Verification items for the finished model (mm, model axes). Face numbers are marked on the shaded views. A direction names the side the tool comes from. Give positions to 0.01 mm unless a question says otherwise; leave off trailing zeros. Order: outer loops, then holes, each group sorted by start corner. A loop starts at its lowest first (then second) coordinate and runs counter-clockwise, first axis right, second up. Notation, with made-up numbers: (16.5, 6.5) -> (70.5, 6.5) arc R22 ccw to (70.5, 13.5) -> close; hole circle Ø3 at (80, 1). An arc over 180 degrees is marked (long way). One line per question, with ' | ' between items. Start each with the question number.
Q1. Access from +Z, -Z, +X, -X, +Y, -Y to the whole of each face (thin tool, end or side, straight path). Record for the marked faces 3, 4 and 5.
Q2. Material ranges on probe 1 along Y at (x, z) = (36.5, 0); probe 2 along Y at (x, z) = (83, 0); probe 3 along X at (y, z) = (14, -23), recorded low to high. Write a range as [from, to].
Q3. Section check A-A on y = 0. Record the cut outline in (x, z), plus the area to 3 significant figures.
Q4. Go/stop test with flat-tipped pins: pin 1 (5 mm diameter, centred on x = 271.5, z = 8.5, fed in from -Y); pin 2 (1.5 mm diameter, centred on x = 93.5, y = 16, fed in from -Z); pin 3 (8 mm diameter, centred on x = 63, y = 22.5, fed in from -Z). Record where each tip stops, or that it passes through.
Q5. Mould release check, pull along Z, two halves, no side actions. Record for the marked faces 1 and 2: released by +Z, released by -Z, zero draft, split by the parting line, or undercut.
Q6. Section check C-C on x = 192.5. Record the cut outline in (y, z).
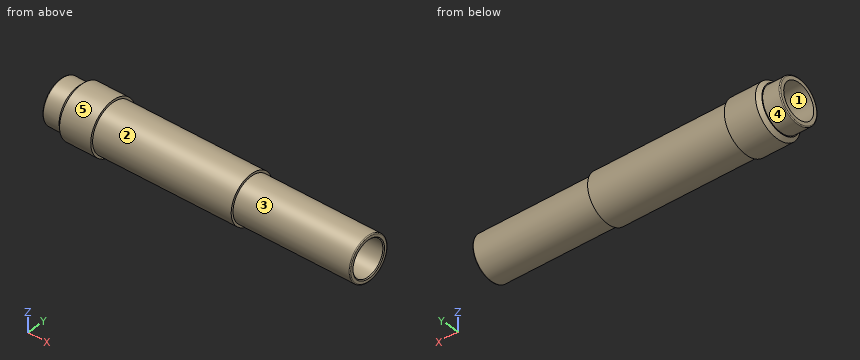
from build123d import *

# Parameters (mm, degrees)
FILLET1_R     = 1
CHAMFER1_SIZE = 1


with BuildPart() as part:
    # Sketch 1 → Revolve3 (revolve)
    with BuildSketch(Plane(origin=(0, 0, 0), x_dir=(1, 0, 0), z_dir=(0, 1, 0)), mode=Mode.PRIVATE) as revolve3_sk:
        Polygon((24, 30), (20, 26), (20, 25), (0, 25), (0, 20), (355, 20), (355, 25), (220, 25), (220, 27.5), (60, 27.5), (60, 30), align=None)
    revolve(revolve3_sk.sketch.rotate(Axis((20, 0, 0), (1, 0, 0)), 180), axis=Axis((20, 0, 0), (1, 0, 0)))

    # Fillet1
    fillet1_edges = [part.edges().sort_by_distance(p)[0] for p in [
        (355, 0, -25),
        (0, 0, -25),
    ]]
    fillet(fillet1_edges, radius=FILLET1_R)

    # Chamfer1
    chamfer1_edges = [part.edges().sort_by_distance(p)[0] for p in [
        (355, 0, -20),
    ]]
    chamfer(chamfer1_edges, length=CHAMFER1_SIZE)


solid = part.part
Filled in:
1) face 3: +X | face 4: -X | face 5: +X, -X
2) probe 1: [-30, -20], [20, 30] | probe 2: [-27.5, -20], [20, 27.5] | probe 3: [20.93, 220]
3) outline: (0, -24) arc R1 ccw to (1, -25) -> (20, -25) -> (20, -26) -> (24, -30) -> (60, -30) -> (60, -27.5) -> (220, -27.5) -> (220, -25) -> (354, -25) arc R1 ccw to (355, -24) -> (355, -21) -> (354, -20) -> (0, -20) -> close; (0, 20) -> (354, 20) -> (355, 21) -> (355, 24) arc R1 ccw to (354, 25) -> (220, 25) -> (220, 27.5) -> (60, 27.5) -> (60, 30) -> (24, 30) -> (20, 26) -> (20, 25) -> (1, 25) arc R1 ccw to (0, 24) -> close | area: 4,730 mm²
4) pin 1: y = -24.27 | pin 2: z = -22.88 | pin 3: z = -22.49
5) face 1: undercut | face 2: split by the parting line
6) outline: circle Ø55 at (0, 0); hole circle Ø40 at (0, 0)
